Here's how the part is built. I have some questions about the finished solid (model axes, mm). Face numbers are marked on the shaded views. Give positions to 0.01 mm unless a question says otherwise; leave off trailing zeros. Loops run counter-clockwise (first coordinate to the right, second up) from the corner with the lowest first, then second, coordinate; pieces in that order, holes last. Notation, with made-up numbers: (-28, 10) - (15, 10) arc R37 cw to (15, 49) - close; hole circle Ø11 at (7.5, 21). An arc over 180 degrees is marked (long way). One line per item, written item: value. Start each with the question number.
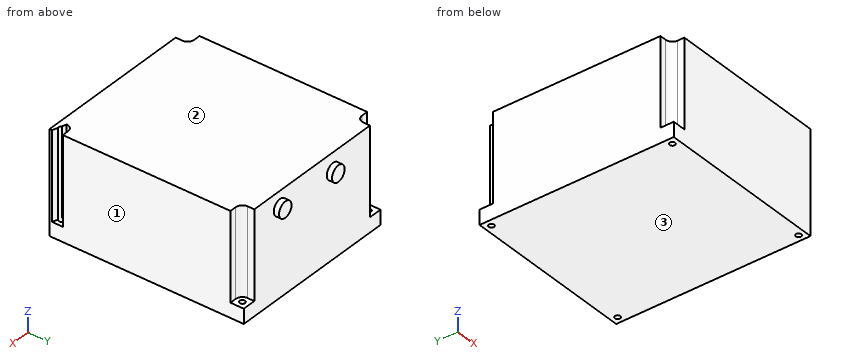
```python
from build123d import *

# Parameters (mm, degrees)
SKETCH1_W           = 130
SKETCH1_H           = 146
SKETCH1_R           = 2
BOSS_EXTRUDE1_DEPTH = 77
CUT_EXTRUDE2_DEPTH  = 66
SKETCH4_R           = 5.985806468
SKETCH4_R_2         = 5.936967647
BOSS_EXTRUDE3_DEPTH = 150


with BuildPart() as part:
    # Sketch1 → Boss-Extrude1 (new body)
    with BuildSketch(Plane.XY):
        with Locations((65, 73)):
            Rectangle(SKETCH1_W, SKETCH1_H)
        with Locations((5, 141)):
            Circle(SKETCH1_R, mode=Mode.SUBTRACT)
        with Locations((125, 141)):
            Circle(SKETCH1_R, mode=Mode.SUBTRACT)
        with Locations((125, 5)):
            Circle(SKETCH1_R, mode=Mode.SUBTRACT)
        with Locations((5, 5)):
            Circle(SKETCH1_R, mode=Mode.SUBTRACT)
    extrude(amount=BOSS_EXTRUDE1_DEPTH)

    # Sketch3 → Cut-Extrude2 (cut)
    with BuildSketch(Plane.XY.offset(77)):
        with BuildLine():
            Line((120, 141), (120, 146))
            Line((120, 146), (146, 160))
            Line((146, 160), (130, 136))
            Line((130, 136), (125, 136))
            ThreePointArc((125, 136), (121.464466094, 137.464466094), (120, 141))
        make_face()
        with BuildLine():
            Line((10, 141), (10, 146))
            Line((10, 146), (0, 160))
            Line((0, 160), (0, 136))
            Line((0, 136), (5, 136))
            ThreePointArc((5, 136), (8.535533906, 137.464466094), (10, 141))
        make_face()
        with BuildLine():
            Line((10, 5), (10, 0))
            Line((10, 0), (0, 0))
            Line((0, 0), (0, 10))
            Line((0, 10), (5, 10))
            ThreePointArc((5, 10), (8.535533906, 8.535533906), (10, 5))
        make_face()
        with BuildLine():
            Line((120, 5), (136, 0))
            Line((136, 0), (146, 0))
            Line((146, 0), (130, 10))
            Line((130, 10), (125, 10))
            ThreePointArc((125, 10), (121.464466094, 8.535533906), (120, 5))
        make_face()
    extrude(amount=-CUT_EXTRUDE2_DEPTH, mode=Mode.SUBTRACT)

    # Sketch4 → Boss-Extrude3 (add)
    with BuildSketch(Plane(origin=(0, 0, 0), x_dir=(-1, 0, 0), z_dir=(0, -1, 0))):
        with Locations(Location((-45.096991408, -63.420422251, 0), (0, 0, 90))):
            Circle(SKETCH4_R)
        with Locations(Location((-95.564941336, -65.16467674, 0), (0, 0, 90))):
            Circle(SKETCH4_R_2)
    extrude(amount=-BOSS_EXTRUDE3_DEPTH)


solid = part.part
```
(1) If we section it at B-B on x = 81: List the corners of the cut face in (y, z) for me.
(2) If we section it at C-C on z = 64: List the corners of the cut face in (x, y) for me (3 decimals), plus the area to 3 significant figures.
(3) If we mould it in two halves opening along Z, with no side actions, what happens to the marked faces 1, 2 and 3? For each: pulls with the +Z half, pulls with the -Z half, needs draft (parallel to the pull), parting line crosses it, or undercut.
(4) If we section it at A-A on z = 27: List the corners of the cut face in (x, y) for me (3 decimals).
(5) Will these pins go through, and if not, where does the flat tip stop? pin 1 (2.5 mm diameter, centred on y = 143.5, z = 30, fed in from +X); pin 2 (2.5 mm diameter, centred on y = 3, z = 44, fed in from -X); pin 3 (3 mm diameter, centred on x = 5, y = 5, fed in from -Z); pin 4 (1 mm diameter, centred on x = 34, z = 9.5, fed in from +Y).
(6) Please list where these lines run through material, in increasing order: probe 1 along Y at (x, z) = (5, 4); probe 2 along X at (y, z) = (141, 5.5); probe 3 along Y at (x, z) = (125, 30). Write a range as from..to.
Found:
1. outline: (0, 0) - (146, 0) - (146, 77) - (0, 77) - close
2. outline: (0, 10) - (5, 10) arc R5 cw to (10, 5) - (10, 0) - (130, 0) - (130, 1.875) - (125.827, 3.179) arc R2 cw to (123.283, 3.974) - (120, 5) arc R5 cw to (125, 10) - (130, 10) - (130, 136) - (125, 136) arc R5 cw to (120, 141) - (120, 146) - (101.387, 146) - (101.387, 150) - (89.743, 150) - (89.743, 146) - (51.055, 146) - (51.055, 150) - (39.139, 150) - (39.139, 146) - (10, 146) - (10, 141) arc R5 cw to (5, 136) - (0, 136) - close
2. area: 18,700 mm^2
3. face 1: needs draft
3. face 2: pulls with the +Z half
3. face 3: pulls with the -Z half
4. outline: (0, 10) - (5, 10) arc R5 cw to (10, 5) - (10, 0) - (130, 0) - (130, 1.875) - (125.827, 3.179) arc R2 cw to (123.283, 3.974) - (120, 5) arc R5 cw to (125, 10) - (130, 10) - (130, 136) - (125, 136) arc R5 cw to (120, 141) - (120, 146) - (10, 146) - (10, 141) arc R5 cw to (5, 136) - (0, 136) - close
5. pin 1: x = 120
5. pin 2: x = 10
5. pin 3: through
5. pin 4: y = 146
6. probe 1: 0..3, 7..139, 143..146
6. probe 2: 0..3, 7..123, 127..130
6. probe 3: 0..3, 10..136
